For this review, use the dimensioned drawing (mm, ordinates from the lowest corner) and the shaded views. A direction names the side the tool comes from. Round coordinates to 2 decimals unless told otherwise and drop trailing zeros. Loops run counter-clockwise (first coordinate to the right, second up) from the corner with the lowest first, then second, coordinate; pieces in that order, holes last. Notation, with made-up numbers: (63, 56) - (80, 56) arc R5 cw to (80, 64) - close; hole circle Ø2 at (39.25, 23.5). An arc over 180 degrees is marked (long way). Use one line per item in the form item = value. Start each with the question number.
(1) We need section B-B, the plane z = 51.5. Write out the cut boundary in (x, y).
(2) We need section C-C, the plane z = 181.5. Write out the cut boundary in (x, y), then the cut area to 3 significant figures.
(3) We need section D-D, the plane x = 62. Write out the cut boundary in (y, z), then the cut area to 3 significant figures.
(4) Wall thickness on probe 1 along Y at (x, z) = (23, 108.5): over which ranges is the line inside the solid? List them lowest first. Write a range as [from, to].
(5) Machinability: for the marked faces 1 and 2, which of the approach directions +Z, -Z, +X, -X, +Y, -Y give a long, thin tool a straight path to every point of the face, cutting with its end or side? Answer none if there is none.
(6) We need section A-A, the plane x = 26. Write out the cut boundary in (y, z).
(7) For pin 1 (1.5 mm diameter, centred on y = 128.5, z = 173, fed in from -X); pin 2 (2 mm diameter, centred on y = 58.5, z = 138, fed in from +X); pin 3 (5 mm diameter, centred on x = 61.5, z = 25, fed in from +Y), all flat-tipped, find the tip position at first contact; note any pin that passes through.
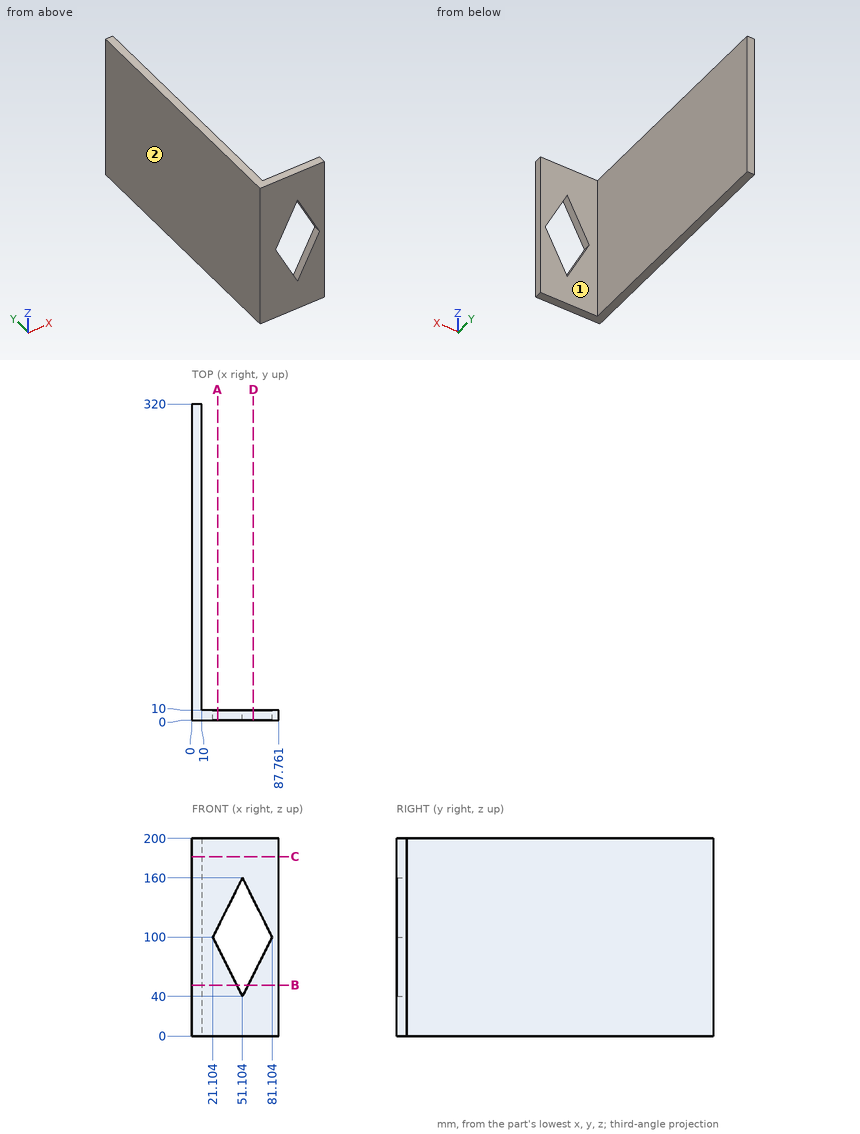
Data:
q1.outline = (0, 0) - (45.35, 0) - (45.35, 10) - (10, 10) - (10, 320) - (0, 320) - close; (56.85, 0) - (87.76, 0) - (87.76, 10) - (56.85, 10) - close
q2.outline = (0, 0) - (87.76, 0) - (87.76, 10) - (10, 10) - (10, 320) - (0, 320) - close
q2.area = 3,980 mm^2
q3.outline = (0, 0) - (10, 0) - (10, 61.79) - (0, 61.79) - close; (0, 138.21) - (10, 138.21) - (10, 200) - (0, 200) - close
q3.area = 1,240 mm^2
q4.probe_1 = [0, 10]
q5.face_1 = +Z, -Z, +X, +Y
q5.face_2 = +Z, -Z, -X, +Y, -Y
q6.outline = (0, 0) - (10, 0) - (10, 90.21) - (0, 90.21) - close; (0, 109.79) - (10, 109.79) - (10, 200) - (0, 200) - close
q7.pin_1 = 0
q7.pin_2 = 10
q7.pin_3 = 10
